Geometry: final body of the model. Coordinates: model frame, mm. A direction names the side the tool comes from. Give positions to 0.01 mm unless a question says otherwise; leave off trailing zeros. Loops run counter-clockwise (first coordinate to the right, second up) from the corner with the lowest first, then second, coordinate; pieces in that order, holes last.
from build123d import *

# Parameters (mm, degrees)
SKETCH1_W                      = 60
SKETCH1_H                      = 50
BOSS_EXTRUDE1_DEPTH            = 30
SKETCH2_W                      = 13.5
SKETCH2_H                      = 40
CUT_EXTRUDE1_DEPTH             = 84.666002653
SKETCH3_W                      = 13.5
SKETCH3_H                      = 40
CUT_EXTRUDE2_DEPTH             = 84.666002653
CUT_EXTRUDE3_DEPTH             = 20
F_9_0_9_DIAMETER_HOLE1_D       = 9
F_10_0_10_DIAMETER_HOLE1_D     = 10
F_10_0_10_DIAMETER_HOLE1_DEPTH = 19
F_10_0_10_DIAMETER_HOLE2_D     = 10
F_10_0_10_DIAMETER_HOLE2_DEPTH = 19


with BuildPart() as part:
    # Sketch1 → Boss-Extrude1 (new body)
    with BuildSketch(Plane.XY.offset(30)):
        with Locations((30, 25)):
            Rectangle(SKETCH1_W, SKETCH1_H)
    extrude(amount=-BOSS_EXTRUDE1_DEPTH)

    # Sketch2 → Cut-Extrude1 (cut, through all)
    with BuildSketch(Plane(origin=(0, 0, 0), x_dir=(-1, 0, 0), z_dir=(0, 0, -1))):
        with Locations((-53.25, 30)):
            Rectangle(SKETCH2_W, SKETCH2_H)
    extrude(amount=-CUT_EXTRUDE1_DEPTH, mode=Mode.SUBTRACT)

    # Sketch3 → Cut-Extrude2 (cut, through all)
    with BuildSketch(Plane(origin=(0, 0, 0), x_dir=(-1, 0, 0), z_dir=(0, 0, -1))):
        with Locations((-6.75, 30)):
            Rectangle(SKETCH3_W, SKETCH3_H)
    extrude(amount=-CUT_EXTRUDE2_DEPTH, mode=Mode.SUBTRACT)

    # Sketch4 → Cut-Extrude3 (cut)
    with BuildSketch(Plane.XY.offset(30)):
        with BuildLine():
            Line((19, 50), (19, 16))
            ThreePointArc((19, 16), (30, 9.437171044), (41, 16))
            Line((41, 16), (41, 50))
            Line((41, 50), (19, 50))
        make_face()
    extrude(amount=-CUT_EXTRUDE3_DEPTH, mode=Mode.SUBTRACT)

    # Ø9.0 (9) Diameter Hole1 (through all)
    with Locations(Plane(origin=(0, 0, 0), x_dir=(-1, 0, 0), z_dir=(0, -1, 0))):
        with Locations((-7.5, -15), (-52.5, -15)):
            Hole(F_9_0_9_DIAMETER_HOLE1_D / 2)

    # Ø10.0 (10) Diameter Hole1
    with Locations(Plane.ZY.offset(-41)):
        with Locations((20, 40)):
            Hole(F_10_0_10_DIAMETER_HOLE1_D / 2, depth=F_10_0_10_DIAMETER_HOLE1_DEPTH)

    # Ø10.0 (10) Diameter Hole2
    with Locations(Plane(origin=(19, 0, 0), x_dir=(0, 0, -1), z_dir=(1, 0, 0))):
        with Locations((-20, 40)):
            Hole(F_10_0_10_DIAMETER_HOLE2_D / 2, depth=F_10_0_10_DIAMETER_HOLE2_DEPTH)


solid = part.part
Item 1: Section query B-B on z = 18.25. Return loops of the section in (x, y), plus the area to 3 significant figures.
Values follow:
outline: (0, 0) - (4.39, 0) - (4.39, 10) - (0, 10) - close; (10.61, 0) - (49.39, 0) - (49.39, 10) - (46.5, 10) - (46.5, 35.32) - (41, 35.32) - (41, 16) arc R12.5 cw to (19, 16) - (19, 35.32) - (13.5, 35.32) - (13.5, 10) - (10.61, 10) - close; (13.5, 44.68) - (19, 44.68) - (19, 50) - (13.5, 50) - close; (41, 44.68) - (46.5, 44.68) - (46.5, 50) - (41, 50) - close; (55.61, 0) - (60, 0) - (60, 10) - (55.61, 10) - close
area: 842 mm2
Item 2: Set-up query: faces 1 (the face through (2, 10, 15)), 2 (the face through (58, 10, 15)), 3 (the face through (19, 33, 20)). Return all of +Z, -Z, +X, -X, +Y, -Y with unobstructed straight access to the full face (end or side cutting, diameter ignored); none if empty.
Values follow:
face 1: +Z, -Z, -X, +Y
face 2: +Z, -Z, +X, +Y
face 3: +Z, +Y
Item 3: Section query A-A on x = 7.5. Return loops of the section in (y, z).
Values follow:
outline: (0, 0) - (10, 0) - (10, 10.5) - (0, 10.5) - close; (0, 19.5) - (10, 19.5) - (10, 30) - (0, 30) - close
Item 4: Section query D-D on z = 8.5. Return loops of the section in (x, y), plus the area to 3 significant figures.
Values follow:
outline: (0, 0) - (60, 0) - (60, 10) - (46.5, 10) - (46.5, 50) - (13.5, 50) - (13.5, 10) - (0, 10) - close
area: 1,920 mm2
Item 5: Pin query (flat end, axial travel): pin 1 (24 mm diameter, centred on x = 29, y = 23, fed in from +Z); pin 2 (10.5 mm diameter, centred on x = 7.5, z = 15, fed in from +Y); pin 3 (10 mm diameter, centred on y = 33.5, z = 23.5, fed in from -X). Return the tip coordinate at first contact, or that it passes through.
Values follow:
pin 1: stops at z = 30
pin 2: stops at y = 10
pin 3: stops at x = 13.5
Item 6: Section query C-C on y = 40. Return loops of the section in (x, z), plus the area to 3 significant figures.
Values follow:
outline: (13.5, 0) - (46.5, 0) - (46.5, 15) - (41, 15) - (41, 10) - (19, 10) - (19, 15) - (13.5, 15) - close; (13.5, 25) - (19, 25) - (19, 30) - (13.5, 30) - close; (41, 25) - (46.5, 25) - (46.5, 30) - (41, 30) - close
area: 440 mm2
Item 7: Ray query, probe 1 along X at (y, z) = (44, 13.25); probe 2 along Z at (x, y) = (7.5, 8.25); probe 3 along X at (y, z) = (46.5, 4). Return the intervals inside material, ascending.
Values follow:
probe 1: x = 13.5 to 19, 41 to 46.5
probe 2: z = 0 to 10.5, 19.5 to 30
probe 3: x = 13.5 to 46.5
Item 8: Draft query along Z for faces 4 (the face through (30, 9, 30)), 5 (the face through (43.788, 44.957, 20.651)), 6 (the face through (30, 50, 9)). Return one class per face: +Z half, -Z half, draft (parallel to the pull), parting line (faces both ways), or undercut.
Values follow:
face 4: +Z half
face 5: undercut
face 6: draft
